Print and shaded views of the part. All mm, measured from the part's lowest x, y and z. A direction names the side the tool comes from. Round coordinates to 2 decimals unless told otherwise and drop trailing zeros. Order: outer loops, then holes, each group sorted by start corner. A loop starts at its lowest first (then second) coordinate and runs counter-clockwise, first axis right, second up.
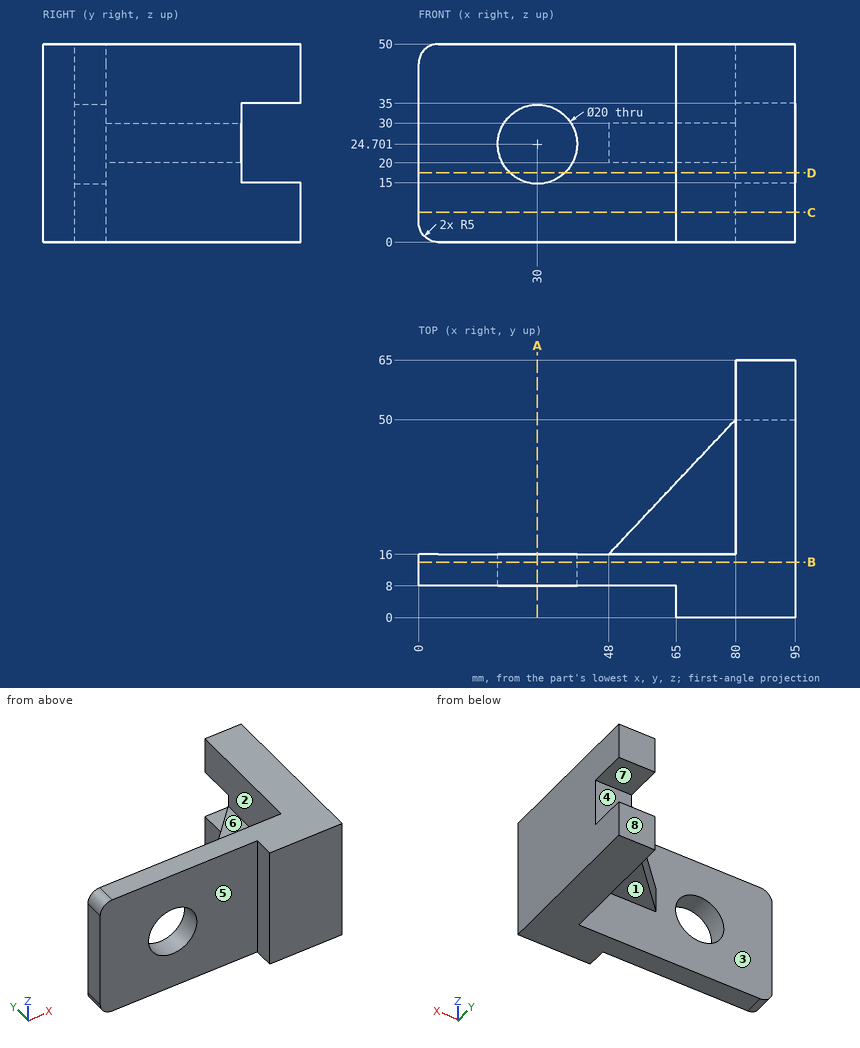
1. Cut at D-D, the plane z = 17.5. Write the cut outline in (x, y), and give its area (3 significant figures).
2. Tool access for the marked faces 1, 2, 3, 4 and 5: list every direction of +Z, -Z, +X, -X, +Y, -Y with a clear straight run to the whole face (end or side of a thin tool).
3. Cut at C-C, the plane z = 7.5. Write the cut outline in (x, y).
4. Mould opens along Z. For the marked faces 6, 7 and 8 say: released by +Z, released by -Z, zero draft, split by the parting line, or undercut.
5. Cut at B-B, the plane y = 14. Write the cut outline in (x, z).
6. Cut at A-A, the plane x = 30. Write the cut outline in (y, z), and give its area (3 significant figures).
7. Drill centre lines: line 1 (Y direction, x = 58, z = 35.5); line 2 (X direction, y = 38.5, z = 3.5); line 3 (Y direction, x = 70, z = 37). Where is each one in solid material? Low to high.
8. Pin check, flat tips, straight feed: P1, Ø1.5, axis at y = 25, z = 42.5, coming from the -X side; P2, Ø12, axis at x = 89.5, z = 23, coming from the +Y side; P3, Ø4, axis at y = 5.5, z = 31, coming from the -X side. Stop position of each tip, or through.
Outcome:
1. outline: (0, 8) - (23.06, 8) - (23.06, 16) - (0, 16) - close; (36.94, 8) - (65, 8) - (65, 0) - (95, 0) - (95, 50) - (80, 50) - (80, 16) - (36.94, 16) - close
1. area: 1,400 mm2
2. face 1: -Z, -X, +Y
2. face 2: +Z, -X, +Y
2. face 3: -X, +Y
2. face 4: +X, -X, +Y
2. face 5: +Z, -Z, -X, -Y
3. outline: (0, 8) - (65, 8) - (65, 0) - (95, 0) - (95, 65) - (80, 65) - (80, 16) - (0, 16) - close
4. face 6: released by +Z
4. face 7: undercut
4. face 8: zero draft
5. outline: (0, 5) arc R5 ccw to (5, 0) - (95, 0) - (95, 50) - (5, 50) arc R5 ccw to (0, 45) - close; hole circle Ø20 at (30, 24.7)
6. outline: (8, 0) - (16, 0) - (16, 14.7) - (8, 14.7) - close; (8, 34.7) - (16, 34.7) - (16, 50) - (8, 50) - close
6. area: 240 mm2
7. line 1: y = 8 to 16
7. line 2: x = 80 to 95
7. line 3: y = 0 to 16
8. P1: stops at x = 80
8. P2: stops at y = 50
8. P3: stops at x = 65
